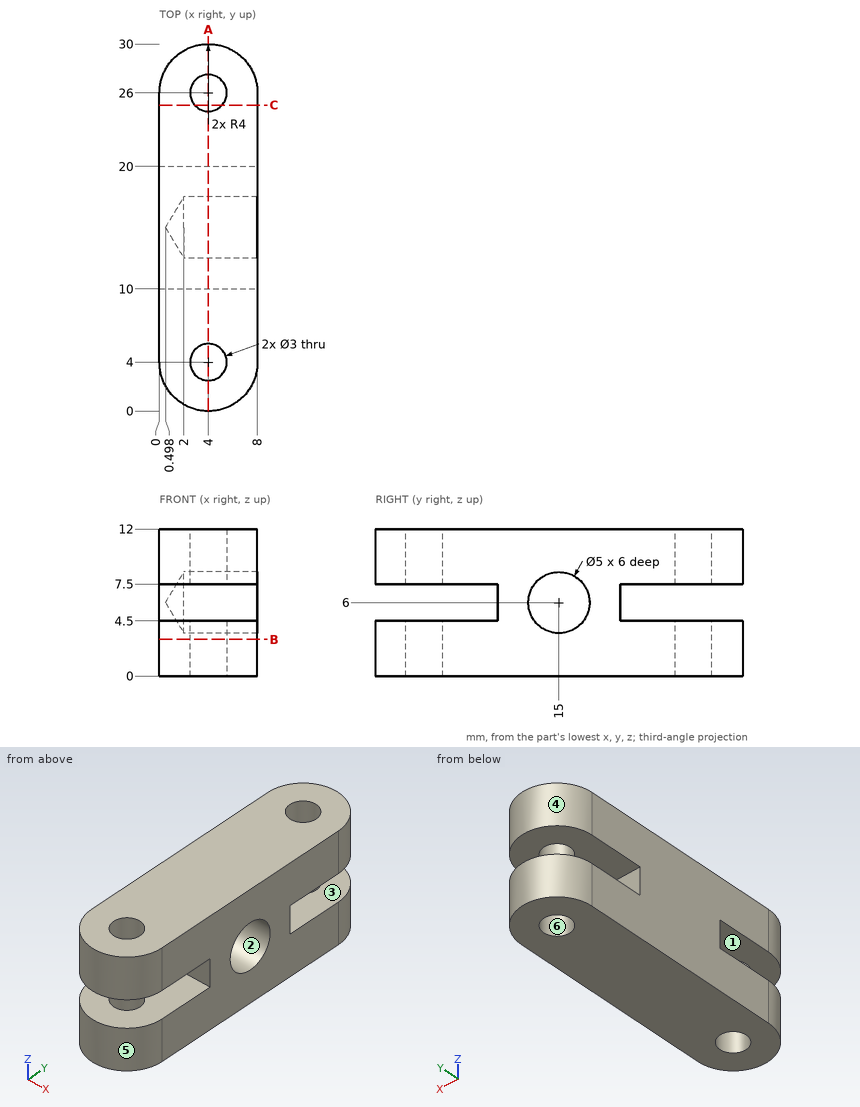
Could you check a few things on this drawing? It's one solid part, dimensions in mm from its lowest x, y, z. A direction names the side the tool comes from. Give positions to 0.01 mm unless a question says otherwise; leave off trailing zeros. Order: outer loops, then holes, each group sorted by start corner. A loop starts at its lowest first (then second) coordinate and runs counter-clockwise, first axis right, second up. Notation, with made-up numbers: (83.5, 1) - (120.5, 1) arc R16 cw to (120.5, 21) - close; hole circle Ø10 at (11.25, -32.5). An arc over 180 degrees is marked (long way). Answer as a JSON object with one key per item and string values. Group by question number.
Item 1: If we section it at C-C on y = 25: Please give me the cut outline in (x, z), and give its area (3 significant figures).
Item 2: If we mould it in two halves opening along Y, with no side actions, what happens to the marked faces 4, 5 and 6? For each: pulls with the +Y half, pulls with the -Y half, needs draft (parallel to the pull), parting line crosses it, or undercut.
Item 3: Please list where these lines run through material, in increasing order: probe 1 along Y at (x, z) = (4, 9.45); probe 2 along Z at (x, y) = (2.75, 2.5); probe 3 along Y at (x, z) = (3.9, 6).
Item 4: If we section it at B-B on z = 3: Please give me the cut outline in (x, y).
Item 5: Which directions (+Z, -Z, +X, -X, +Y, -Y) give clear straight access to the entire face, cutting with the end or side of a thin tool? Please do the marked faces 1, 2 and 3.
Item 6: For P1, Ø1, axis at x = 5.5, z = 6, coming from the -Y side; P2, Ø4, axis at x = 6, z = 5.5, coming from the -Y side; P3, Ø0.9, axis at x = 4.5, z = 6.5, coming from the +Y side, each with a flat end and sliding along its axis, tell me the tip position at first contact or that it passes through.
Item 7: If we section it at A-A on x = 4: Give the number of separate pieces and of enclosed holes in the cut face, and give its area (3 significant figures).
Result set:
{
 "1": {"outline": "(0, 0) - (2.88, 0) - (2.88, 4.5) - (0, 4.5) - close; (0, 7.5) - (2.88, 7.5) - (2.88, 12) - (0, 12) - close; (5.12, 0) - (8, 0) - (8, 4.5) - (5.12, 4.5) - close; (5.12, 7.5) - (8, 7.5) - (8, 12) - (5.12, 12) - close", "area": "51.9 mm²"},
 "2": {"face 4": "pulls with the +Y half", "face 5": "pulls with the -Y half", "face 6": "undercut"},
 "3": {"probe 1": "0 to 2.5, 5.5 to 24.5, 27.5 to 30", "probe 2": "0 to 4.5, 7.5 to 12", "probe 3": "10 to 12.5, 17.5 to 20"},
 "4": {"outline": "(0, 4) arc R4 ccw to (8, 4) - (8, 26) arc R4 ccw to (0, 26) - close; hole circle Ø3 at (4, 4); hole circle Ø3 at (4, 26)"},
 "5": {"face 1": "+X, -X, -Y", "face 2": "+X", "face 3": "+X, -X, +Y"},
 "6": {"P1": "y = 10", "P2": "y = 0.01", "P3": "y = 20"},
 "7": {"separate pieces": "5", "enclosed holes": "1", "area": "226 mm²"}
}
